Part model, mm, in its own coordinate system. Face numbers are marked on the shaded views. A direction names the side the tool comes from. Coordinates: 2 decimals unless noted, no trailing zeros. Loops run counter-clockwise (first coordinate to the right, second up) from the corner with the lowest first, then second, coordinate; pieces in that order, holes last. Notation, with made-up numbers: (-22, -38.5) -> (13, -38.5) arc R34 ccw to (13, -7.5) -> close; hole circle Ø9 at (14, -10). An arc over 180 degrees is marked (long way). One line per item, written item: value. Start each with the question number.
from build123d import *

# Parameters (mm, degrees)
BASE_PLATE_SKETCH_W        = 92
BASE_PLATE_SKETCH_H        = 36
BASE_PLATE_DEPTH           = 8
ROUNDED_ENDS_R18_DEPTH     = 8
UPRIGHT_LEG_DEPTH          = 10
LUG_HEAD_DEPTH             = 10
RAISED_START               = 10
ROUND_BOSS_SKETCH_R        = 15
RAISED_ROUND_BOSS_30_DEPTH = 10
BOSS_BORE_SKETCH_R         = 10
BOSS_BORE_20_DEPTH         = 20
MOUNTING_HOLES_SKETCH_R    = 8
MOUNTING_HOLES_2X_16_DEPTH = 20
RIB_DEPTH                  = 40
RIB_TRIM_CUT_1_DEPTH       = 14
RIB_TRIM_CUT_2_DEPTH       = 14


with BuildPart() as part:
    # Base Plate Sketch → Base Plate (new body)
    with BuildSketch(Plane.XY):
        with Locations((46, 18)):
            Rectangle(BASE_PLATE_SKETCH_W, BASE_PLATE_SKETCH_H)
    extrude(amount=BASE_PLATE_DEPTH)

    # Rounded Ends Sketch → Rounded Ends R18 (cut)
    with BuildSketch(Plane.XY.offset(8)):
        with BuildLine():
            Line((18, 36), (0, 36))
            Line((0, 36), (0, 18))
            ThreePointArc((0, 18), (5.272077939, 30.727922061), (18, 36))
        make_face()
        with BuildLine():
            ThreePointArc((18, 0), (5.272077939, 5.272077939), (0, 18))
            Line((0, 18), (0, 0))
            Line((0, 0), (18, 0))
        make_face()
        with BuildLine():
            Line((92, 0), (92, 18))
            ThreePointArc((92, 18), (86.727922061, 5.272077939), (74, 0))
            Line((74, 0), (92, 0))
        make_face()
        with BuildLine():
            Line((92, 36), (74, 36))
            ThreePointArc((74, 36), (86.727922061, 30.727922061), (92, 18))
            Line((92, 18), (92, 36))
        make_face()
    extrude(amount=-ROUNDED_ENDS_R18_DEPTH, mode=Mode.SUBTRACT)

    # Upright Leg Sketch → Upright Leg (add)
    with BuildSketch(Plane(origin=(0, 36, 0), x_dir=(1, 0, 0), z_dir=(0, 1, 0))):
        Polygon((46, 0), (26, 0), (26, 32), (66, 32), (66, 0), align=None)
    extrude(amount=-UPRIGHT_LEG_DEPTH)

    # Lug Head Sketch → Lug Head (add)
    with BuildSketch(Plane(origin=(0, 0, -32), x_dir=(-1, 0, 0), z_dir=(0, 0, -1))):
        with BuildLine():
            Line((-66, 36), (-26, 36))
            Line((-26, 36), (-31.189048708, 68.373967528))
            ThreePointArc((-31.189048708, 68.373967528), (-46, 81), (-60.810951292, 68.373967528))
            Line((-60.810951292, 68.373967528), (-66, 36))
        make_face()
    extrude(amount=-LUG_HEAD_DEPTH)

    # Round Boss Sketch → Raised Round Boss Ø30 (add)
    with BuildSketch(Plane(origin=(0, 0, -32), x_dir=(-1, 0, 0), z_dir=(0, 0, -1)).offset(RAISED_START)):
        with Locations((-46, 66)):
            Circle(ROUND_BOSS_SKETCH_R)
    extrude(amount=-RAISED_ROUND_BOSS_30_DEPTH)

    # Boss Bore Sketch → Boss Bore Ø20 (cut)
    with BuildSketch(Plane(origin=(0, 0, -42), x_dir=(-1, 0, 0), z_dir=(0, 0, -1))):
        with Locations((-46, 66)):
            Circle(BOSS_BORE_SKETCH_R)
    extrude(amount=-BOSS_BORE_20_DEPTH, mode=Mode.SUBTRACT)

    # Mounting Holes Sketch → Mounting Holes 2xØ16 (cut)
    with BuildSketch(Plane(origin=(0, 0, 0), x_dir=(-1, 0, 0), z_dir=(0, 0, -1))):
        with Locations((-74, 18)):
            Circle(MOUNTING_HOLES_SKETCH_R)
        with Locations((-18, 18)):
            Circle(MOUNTING_HOLES_SKETCH_R)
    extrude(amount=-MOUNTING_HOLES_2X_16_DEPTH, mode=Mode.SUBTRACT)

    # Rib Sketch → Rib (add)
    with BuildSketch(Plane.ZY.offset(-26)):
        Polygon((-32, 26), (0, 26), (0, 0), align=None)
    extrude(amount=-RIB_DEPTH)

    # Rib Trim Sketch 1 → Rib Trim Cut 1 (cut)
    with BuildSketch(Plane.ZY.offset(-26)):
        Polygon((-32, 26), (0, 26), (0, 0), align=None)
    extrude(amount=-RIB_TRIM_CUT_1_DEPTH, mode=Mode.SUBTRACT)

    # Rib Trim Sketch 2 → Rib Trim Cut 2 (cut)
    with BuildSketch(Plane(origin=(66, 0, 0), x_dir=(0, 0, -1), z_dir=(1, 0, 0))):
        Polygon((32, 26), (0, 26), (0, 0), align=None)
    extrude(amount=-RIB_TRIM_CUT_2_DEPTH, mode=Mode.SUBTRACT)


solid = part.part
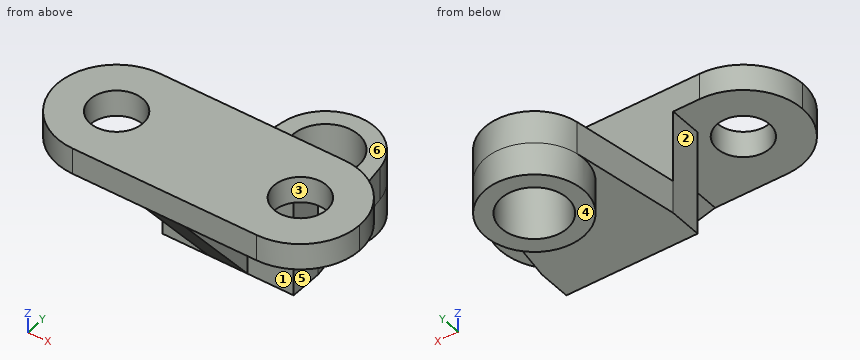
1) Probe line 1 (Y direction, x = 18, z = 2.5); line 2 (Y direction, x = 46, z = -35.25); line 3 (Z direction, x = 40, y = 26.5). List the from-to ranges inside material, lowest first. Write a range as from..to.
2) Pin check, flat tips, straight feed: pin 1 Ø13 at (y, z) = (11.5, -15) entering from +X; pin 2 Ø13 at (x, y) = (18, 18) entering from -Z; pin 3 Ø7 at (x, z) = (56, -10.5) entering from -Y; pin 4 Ø12 at (x, y) = (17, 15) entering from -Z. Stop position of each tip, or through.
3) Slice it at B-B (y = 13). Give the cut face in (x, z) (3 decimals).
4) Slice it at C-C (y = 59.5). Give the cut face in (x, z).
5) Tool access for the marked faces 4, 5 and 6: list every direction of +Z, -Z, +X, -X, +Y, -Y with a clear straight run to the whole face (end or side of a thin tool).
6) Slice it at D-D (z = -14). Give the cut face in (x, y) (3 decimals), then the cut area to 4 significant figures.
7) Pull direction Y, two halves, no side cores. Call the marked faces 1, 2 and 3: +Y half, -Y half, draft (parallel to the pull), parting line (faces both ways), or undercut.
8) Slice it at A-A (x = 46). Give the cut face in (y, z), then the cut area to 3 significant figures.
Check sheet entries:
1. line 1: y = 0..10, 26..36
1. line 2: y = 51..56, 76..81
1. line 3: z = -32..8
2. pin 1: stops at x = 52
2. pin 2: passes through
2. pin 3: stops at y = 26
2. pin 4: stops at z = 0
3. outline: (0.708, 0) -> (11.755, 0) -> (11.755, 8) -> (0.708, 8) -> close; (24.245, 0) -> (40, 0) -> (40, -16) -> (52, -16) -> (52, 0) -> (67.755, 0) -> (67.755, 8) -> (24.245, 8) -> close; (80.245, 0) -> (91.292, 0) -> (91.292, 8) -> (80.245, 8) -> close
4. outline: (29.77, -32) -> (32.48, -32) -> (32.48, -42) -> (38.4, -42) -> (38.4, -22) -> (29.77, -22) -> close; (53.6, -42) -> (59.52, -42) -> (59.52, -32) -> (62.23, -32) -> (62.23, -22) -> (53.6, -22) -> close
5. face 4: -Z, +X, -X, +Y, -Y
5. face 5: -Z, +X, +Y, -Y
5. face 6: +Z, +X, -X, +Y
6. outline: (26, 26) -> (40, 26) -> (40, 11.375) -> (52, 11.375) -> (52, 26) -> (66, 26) -> (66, 36) -> (26, 36) -> close
6. area: 575.5 mm^2
7. face 1: -Y half
7. face 2: draft
7. face 3: undercut
8. outline: (0, 0) -> (26, -32) -> (51, -32) -> (51, -42) -> (56, -42) -> (56, -22) -> (36, -22) -> (36, 8) -> (0, 8) -> close; (76, -42) -> (81, -42) -> (81, -22) -> (76, -22) -> close
8. area: 1,370 mm^2
